from build123d import *

# Parameters (mm, degrees)
BOSS_EXTRUDE1_DEPTH       = 26
CHAMFER1_SIZE             = 2
M8X1_0_TAPPED_HOLE1_D     = 7
M8X1_0_TAPPED_HOLE1_DEPTH = 11
M8X1_0_TAPPED_HOLE1_TIP   = 2.103012167
HOLE2_D                   = 9
SKETCH11_R                = 32.5
CUT_EXTRUDE1_DEPTH        = 2.5
CUT_EXTRUDE2_START        = -2.5
SKETCH12_R                = 32.5
CUT_EXTRUDE2_DEPTH        = 2.5
HOLE3_D                   = 4


with BuildPart() as part:
    # Sketch1 → Boss-Extrude1 (new body)
    with BuildSketch(Plane.XY):
        with BuildLine():
            Line((-50, 24), (-33, 24))
            Line((-33, 24), (-33, 47))
            Line((-33, 47), (33, 47))
            Line((33, 47), (33, 24))
            Line((33, 24), (50, 24))
            Line((50, 24), (50, 0))
            Line((50, 0), (30, 0))
            ThreePointArc((30, 0), (0, 30), (-30, 0))
            Line((-30, 0), (-50, 0))
            Line((-50, 0), (-50, 24))
        make_face()
    extrude(amount=BOSS_EXTRUDE1_DEPTH)

    # Chamfer1
    chamfer1_edges = [part.edges().sort_by_distance(p)[0] for p in [
        (-50, 24, 13),
        (-33, 47, 13),
        (33, 47, 13),
        (50, 24, 13),
    ]]
    chamfer(chamfer1_edges, length=CHAMFER1_SIZE)

    # M8x1.0 Tapped Hole1
    with Locations(Plane(origin=(0, 47, 0), x_dir=(1, 0, 0), z_dir=(0, 1, 0))):
        with Locations((0, -13)):
            Hole(M8X1_0_TAPPED_HOLE1_D / 2, depth=M8X1_0_TAPPED_HOLE1_DEPTH)
            with Locations((0, 0, -(M8X1_0_TAPPED_HOLE1_DEPTH + M8X1_0_TAPPED_HOLE1_TIP / 2))):  # 118° drill point
                Cone(0, M8X1_0_TAPPED_HOLE1_D / 2, M8X1_0_TAPPED_HOLE1_TIP, mode=Mode.SUBTRACT)

    # Hole2 (through all)
    with Locations(Plane(origin=(0, 24, 0), x_dir=(1, 0, 0), z_dir=(0, 1, 0))):
        with Locations((-41, -13), (41, -13)):
            Hole(HOLE2_D / 2)

    # Sketch11 → Cut-Extrude1 (cut)
    with BuildSketch(Plane.XY.offset(26)):
        Circle(SKETCH11_R)
    extrude(amount=-CUT_EXTRUDE1_DEPTH, mode=Mode.SUBTRACT)

    # Sketch12 → Cut-Extrude2 (cut)
    with BuildSketch(Plane(origin=(0, 0, 0), x_dir=(-1, 0, 0), z_dir=(0, 0, -1)).offset(CUT_EXTRUDE2_START)):
        Circle(SKETCH12_R)
    extrude(amount=CUT_EXTRUDE2_DEPTH, mode=Mode.SUBTRACT)

    # Hole3 (through all)
    with Locations(Plane(origin=(0, 47, 0), x_dir=(1, 0, 0), z_dir=(0, 1, 0))):
        with Locations((0, -13)):
            Hole(HOLE3_D / 2)


solid = part.part
Can you work these out from the model? Positions are in its coordinate system, mm. A direction names the side the tool comes from. Give positions to 0.01 mm unless a question says otherwise; leave off trailing zeros. Write each loop counter-clockwise with the first axis right and the second up, starting at its lowest first coordinate (ties: lowest second). Pieces come first, ordered by that corner, then holes. Notation, with made-up numbers: (59, -14) -> (88, -14) arc R20 cw to (88, -10) -> close; hole circle Ø5 at (20, -16.75). An arc over 180 degrees is marked (long way). Answer as a JSON object with one key per item and string values. Group by question number.
Item 1: I'm going to push flat-ended pins straight in: P1, Ø1.5, axis at y = 38, z = 19, coming from the -X side; P2, Ø10.5, axis at y = 39.5, z = 15.5, coming from the +X side; P3, Ø12, axis at x = 37.5, z = 18, coming from the +Y side. Where does each tip first touch, or does it pass through?
Item 2: Suppose I cut it at C-C (x = -41). Please give me the cut outline in (y, z).
Item 3: Please list where these lines run through material, in increasing order: line 1 (Z direction, x = -41, y = 5); line 2 (X direction, y = 44, z = 13); line 3 (X direction, y = 32.25, z = 13). Write a range as [from, to].
Item 4: Suppose I cut it at A-A (z = 13). State how many separate pieces and enclosed holes the cut face has, plus the area to 3 significant figures.
Item 5: For faces 1 (the face through (33, 35, 13)), 2 (the face through (0.715, 32.492, 24.768)), 3 (the face through (0, 31, 2.5)), 4 (the face through (0.759, 41.423, 16.417)), which set-ups out of +Z, -Z, +X, -X, +Y, -Y let a thin tool reach every point of the face, with its end or its side?
Item 6: Suppose I cut it at D-D (y = 33.5). Please give me the cut outline in (x, z), plus the area to 3 significant figures.
Item 7: Suppose I cut it at B-B (y = 17). Please give me the cut outline in (x, z), plus the area to 3 significant figures.
Item 8: We'd pull the mould along X, two halves only. Please class faces 5 (the face through (-37, 24, 10)), 6 (the face through (-50, 11, 13)), 7 (the face through (-0.715, 32.492, 1.268)): +X half, -X half, draft (parallel to the pull), parting line (faces both ways), or undercut.
Findings:
{
 "1": {"P1": "stops at x = -33", "P2": "stops at x = 33", "P3": "stops at y = 46.5"},
 "2": {"outline": "(0, 0) -> (24, 0) -> (24, 8.5) -> (0, 8.5) -> close; (0, 17.5) -> (24, 17.5) -> (24, 26) -> (0, 26) -> close"},
 "3": {"line 1": "z = [0, 8.5], [17.5, 26]", "line 2": "x = [-33, -3.5], [3.5, 33]", "line 3": "x = [-33, -2], [2, 33]"},
 "4": {"separate pieces": "4", "enclosed holes": "0", "area": "1,960 mm²"},
 "5": {"face 1": "+Z, -Z, +X, +Y", "face 2": "+Z, -Y", "face 3": "-Z, -Y", "face 4": "+Y"},
 "6": {"outline": "(-33, 0) -> (33, 0) -> (33, 26) -> (-33, 26) -> close; hole circle Ø4 at (0, 13)", "area": "1,700 mm²"},
 "7": {"outline": "(-50, 0) -> (-27.7, 0) -> (-27.7, 2.5) -> (-24.72, 2.5) -> (-24.72, 23.5) -> (-27.7, 23.5) -> (-27.7, 26) -> (-50, 26) -> close; (24.72, 2.5) -> (27.7, 2.5) -> (27.7, 0) -> (50, 0) -> (50, 26) -> (27.7, 26) -> (27.7, 23.5) -> (24.72, 23.5) -> close; hole circle Ø9 at (-41, 13); hole circle Ø9 at (41, 13)", "area": "1,160 mm²"},
 "8": {"face 5": "draft", "face 6": "-X half", "face 7": "undercut"}
}
